The model under review builds one solid part; all positions refer to its coordinate system, in mm. Face numbers are marked on the shaded views. A direction names the side the tool comes from. Coordinates: 2 decimals unless noted, no trailing zeros. Order: outer loops, then holes, each group sorted by start corner. A loop starts at its lowest first (then second) coordinate and runs counter-clockwise, first axis right, second up. Notation, with made-up numbers: M 83.25,65.25 L 116.25,65.25 A4 cw 116.25,72.25 Z; hole C -6,-23 d2. An arc over 180 degrees is marked long. One line per item, written item: value.
```python
from build123d import *

# Parameters (mm, degrees)
SKETCH_1_4_R        = 75
BOSS_EXTRUDE1_DEPTH = 18
SKETCH_1_3_R        = 50
BOSS_EXTRUDE2_DEPTH = 100
BOSS_EXTRUDE3_START = -118
SKETCH_1_4_2_R      = 75
BOSS_EXTRUDE3_DEPTH = 18


with BuildPart() as part:
    # Sketch 1_4 → Boss-Extrude1 (new body)
    with BuildSketch(Plane(origin=(0, 0, 0), x_dir=(0, 0, -1), z_dir=(1, 0, 0))):
        Circle(SKETCH_1_4_R)
    extrude(amount=BOSS_EXTRUDE1_DEPTH)

    # 草图1<3> → Boss-Extrude2 (add)
    with BuildSketch(Plane(origin=(0, 0, 0), x_dir=(0, 0, -1), z_dir=(1, 0, 0))):
        Circle(SKETCH_1_3_R)
    extrude(amount=-BOSS_EXTRUDE2_DEPTH)

    # Sketch 1_4 2 → Boss-Extrude3 (add)
    with BuildSketch(Plane(origin=(0, 0, 0), x_dir=(0, 0, -1), z_dir=(1, 0, 0)).offset(BOSS_EXTRUDE3_START)):
        Circle(SKETCH_1_4_2_R)
    extrude(amount=BOSS_EXTRUDE3_DEPTH)


solid = part.part
```
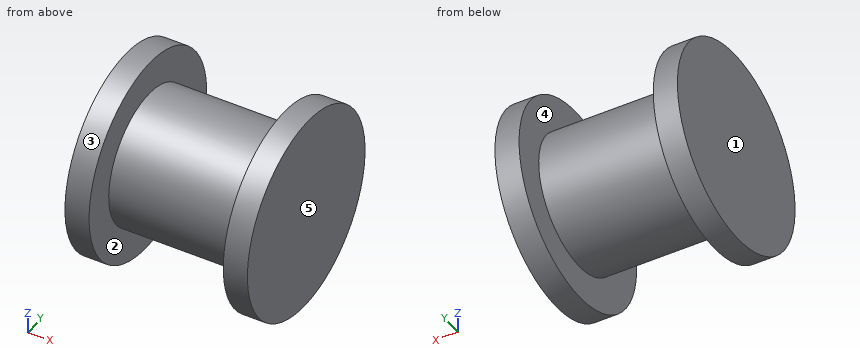
(1) Mouldability with a two-part tool opening along X and no side actions: class the marked faces 3, 4 and 5 as +X half, -X half, draft (parallel to the pull), parting line (faces both ways), or undercut.
Geometry results:
face 3: draft
face 4: undercut
face 5: +X half
(2) For L1, parallel to X at y = -67, z = 16; L2, parallel to Z at x = -2, y = -26.5; L3, parallel to Z at x = 2, y = -64.5, list the stretches that pass through material, from the lowest coordinate up.
Geometry results:
L1: x = -118 to -100, 0 to 18
L2: z = -42.4 to 42.4
L3: z = -38.27 to 38.27
(3) We need section C-C, the plane z = 56.5. State the section outline as (x, y) points.
Geometry results:
outline: M -118,-49.32 L -100,-49.32 L -100,49.32 L -118,49.32 Z; M 0,-49.32 L 18,-49.32 L 18,49.32 L 0,49.32 Z
(4) Insertion check: pin 1 Ø1 at (x, y) = (-75.5, 45.5) entering from -Z; pin 2 Ø8 at (x, z) = (-101.5, 40) entering from +Y; pin 3 Ø6 at (x, y) = (-31.5, -23) entering from +Z. Each pin has a flat end and moves straight along its axis. Give the tip position at first contact, or say it passes through.
Geometry results:
pin 1: stops at z = -21.79
pin 2: stops at y = 65.8
pin 3: stops at z = 45.83
(5) Tool access review of the marked faces 1 and 2: name each direction out of +Z, -Z, +X, -X, +Y, -Y from which nothing blocks a thin tool from reaching the whole face with its end or side.
Geometry results:
face 1: +Z, -Z, -X, +Y, -Y
face 2: none
(6) We need section D-D, the plane x = 4.5. State the section outline as (y, z) points.
Geometry results:
outline: C 0,0 d150
(7) We need section A-A, the plane y = 0. State the section outline as (x, z) points.
Geometry results:
outline: M -118,-75 L -100,-75 L -100,-50 L 0,-50 L 0,-75 L 18,-75 L 18,75 L 0,75 L 0,50 L -100,50 L -100,75 L -118,75 Z
